```python
from build123d import *

# Parameters (mm, degrees)
SKETCH1_W           = 100
SKETCH1_H           = 14
BOSS_EXTRUDE1_DEPTH = 30
SKETCH2_R           = 11
CUT_EXTRUDE1_DEPTH  = 105.637469388
CHAMFER1_SIZE       = 1


with BuildPart() as part:
    # Sketch1 → Boss-Extrude1 (new body)
    with BuildSketch(Plane.XY):
        Rectangle(SKETCH1_W, SKETCH1_H)
    extrude(amount=BOSS_EXTRUDE1_DEPTH)

    # Sketch2 → Cut-Extrude1 (cut, through all)
    with BuildSketch(Plane.ZY.offset(50)):
        with Locations((15, -8)):
            Circle(SKETCH2_R)
    extrude(amount=-CUT_EXTRUDE1_DEPTH, mode=Mode.SUBTRACT)

    # Chamfer1
    chamfer1_edges = [part.edges().sort_by_distance(p)[0] for p in [
        (0, 7, 0),
        (0, 7, 30),
    ]]
    chamfer(chamfer1_edges, length=CHAMFER1_SIZE)


solid = part.part
```
The model under review builds one solid part; all positions refer to its coordinate system, in mm. Give positions to 0.01 mm unless a question says otherwise; leave off trailing zeros. Write each loop counter-clockwise with the first axis right and the second up, starting at its lowest first coordinate (ties: lowest second). Pieces come first, ordered by that corner, then holes.
(1) Consider section D-D, the plane z = 9. Give the boundary of the cut face in (x, y), and give its area (3 significant figures).
(2) Consider section C-C, the plane y = 2. Give the boundary of the cut face in (x, z), and give its area (3 significant figures).
(3) The part is to be moulded in two halves that separate along Z. For faces 1 (the flat face through (-1, 0, 30)), 2 (the flat face through (-1, 0, 0)), 3 (the cylindrical face through (-1, 3, 15)), say which applies: released by +Z, released by -Z, zero draft, split by the parting line, or undercut.
(4) To check wall thickness, follow L1, parallel to Z at x = -24, y = 1.25; L2, parallel to Z at x = -34, y = -0.25; L3, parallel to Y at x = 2.5, z = 16. State the ranges of each line that lie inside material, in increasing order.
(5) Consider section A-A, the plane y = -4.5. Give the boundary of the cut face in (x, z).
(6) For P1, Ø2, axis at x = 3, z = 20, coming from the -Y side; P2, Ø8, axis at y = -3.5, z = 5.5, coming from the -X side; P3, Ø2, axis at x = 38.5, z = 14, coming from the -Y side; P4, Ø5, axis at x = -8, z = 15, coming from the -Y side, all flat-tipped, find the tip position at first contact; note any pin that passes through.
(7) Consider section B-B, the plane x = 14. Give the boundary of the cut face in (y, z), and give its area (3 significant figures).
Returned:
1. outline: (-50, 1.22) - (50, 1.22) - (50, 7) - (-50, 7) - close
1. area: 578 mm2
2. outline: (-50, 0) - (50, 0) - (50, 10.42) - (-50, 10.42) - close; (-50, 19.58) - (50, 19.58) - (50, 30) - (-50, 30) - close
2. area: 2,080 mm2
3. face 1: released by +Z
3. face 2: released by -Z
3. face 3: undercut
4. L1: z = 0 to 9.05, 20.95 to 30
4. L2: z = 0 to 7.19, 22.81 to 30
4. L3: y = 2.95 to 7
5. outline: (-50, 0) - (50, 0) - (50, 4.57) - (-50, 4.57) - close; (-50, 25.43) - (50, 25.43) - (50, 30) - (-50, 30) - close
6. P1: stops at y = 1.22
6. P2: stops at x = -50
6. P3: stops at y = 2.82
6. P4: stops at y = 2.71
7. outline: (-7, 0) - (6, 0) - (7, 1) - (7, 29) - (6, 30) - (-7, 30) - (-7, 25.95) arc R11 cw to (-7, 4.05) - close
7. area: 251 mm2
